Study the drawing (mm; zero at the part's minimum x, y, z) and answer. Round coordinates to 2 decimals unless told otherwise and drop trailing zeros. Loops run counter-clockwise (first coordinate to the right, second up) from the corner with the lowest first, then second, coordinate; pieces in that order, holes last. Notation, with made-up numbers: (24.25, 14.25) -> (33.25, 14.25) arc R23 cw to (33.25, 46.25) -> close; hole circle Ø11 at (-37.75, 30). An arc over 180 degrees is marked (long way). Use one line per item in the form item = value.
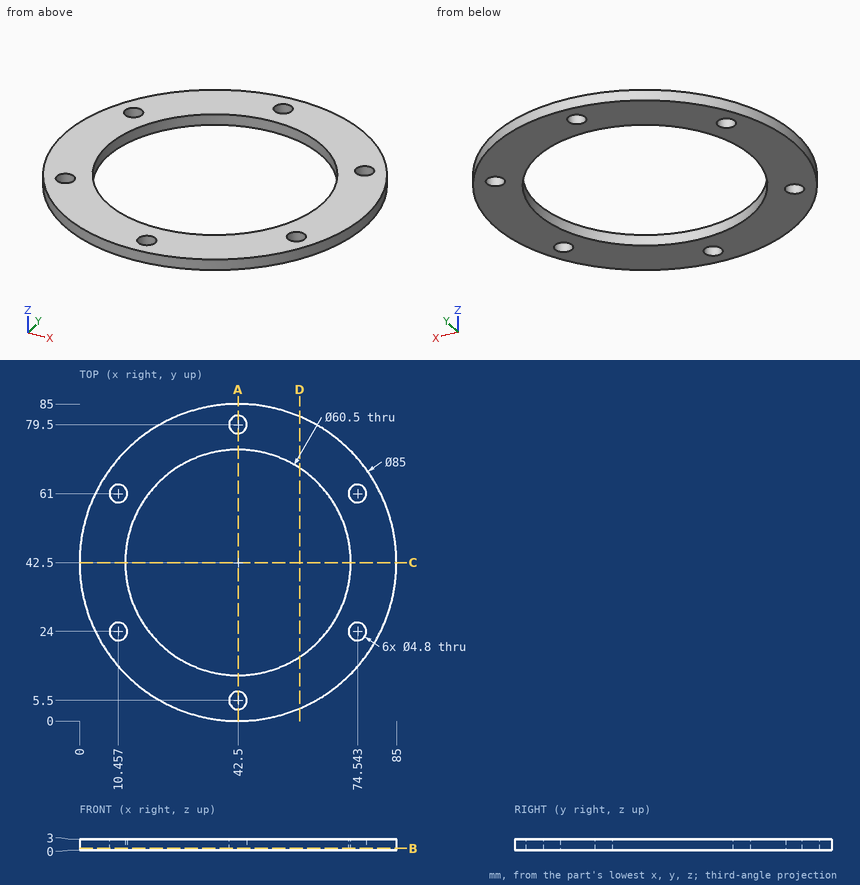
(1) Find section D-D, the plane x = 59. Write down the section's boundary in (y, z), then the cut area to 3 significant figures.
Completed:
outline = (3.33, 0) -> (17.15, 0) -> (17.15, 3) -> (3.33, 3) -> close; (67.85, 0) -> (81.67, 0) -> (81.67, 3) -> (67.85, 3) -> close
area = 82.9 mm2
(2) Find section B-B, the plane z = 0.5. Write down the section's boundary in (x, y), then the cut area to 3 significant figures.
Completed:
outline = circle Ø85 at (42.5, 42.5); hole circle Ø4.8 at (10.46, 24); hole circle Ø4.8 at (10.46, 61); hole circle Ø60.5 at (42.5, 42.5); hole circle Ø4.8 at (42.5, 5.5); hole circle Ø4.8 at (42.5, 79.5); hole circle Ø4.8 at (74.54, 24); hole circle Ø4.8 at (74.54, 61)
area = 2,690 mm2
(3) Consider L1, parallel to Y at x = 42.5, z = 2.25; L2, parallel to X at y = 25.5, z = 1.2; L3, parallel to Y at x = 59, z = 0.85. Determine where each line is inside the solid, lowest interval first.
Completed:
L1 = 0 to 3.1, 7.9 to 12.25, 72.75 to 77.1, 81.9 to 85
L2 = 3.55 to 8.58, 12.33 to 17.48, 67.52 to 72.67, 76.42 to 81.45
L3 = 3.33 to 17.15, 67.85 to 81.67
(4) Find section A-A, the plane x = 42.5. Write down the section's boundary in (y, z), then the cut area to 3 significant figures.
Completed:
outline = (0, 0) -> (3.1, 0) -> (3.1, 3) -> (0, 3) -> close; (7.9, 0) -> (12.25, 0) -> (12.25, 3) -> (7.9, 3) -> close; (72.75, 0) -> (77.1, 0) -> (77.1, 3) -> (72.75, 3) -> close; (81.9, 0) -> (85, 0) -> (85, 3) -> (81.9, 3) -> close
area = 44.7 mm2
(5) Find section C-C, the plane y = 42.5. Write down the section's boundary in (x, z).
Completed:
outline = (0, 0) -> (12.25, 0) -> (12.25, 3) -> (0, 3) -> close; (72.75, 0) -> (85, 0) -> (85, 3) -> (72.75, 3) -> close
